Job drawing, mm, ordinate dimensions from the low corner. One solid piece. A direction names the side the tool comes from. Coordinates: 2 decimals unless noted, no trailing zeros. Write each loop counter-clockwise with the first axis right and the second up, starting at its lowest first coordinate (ties: lowest second). Pieces come first, ordered by that corner, then holes.
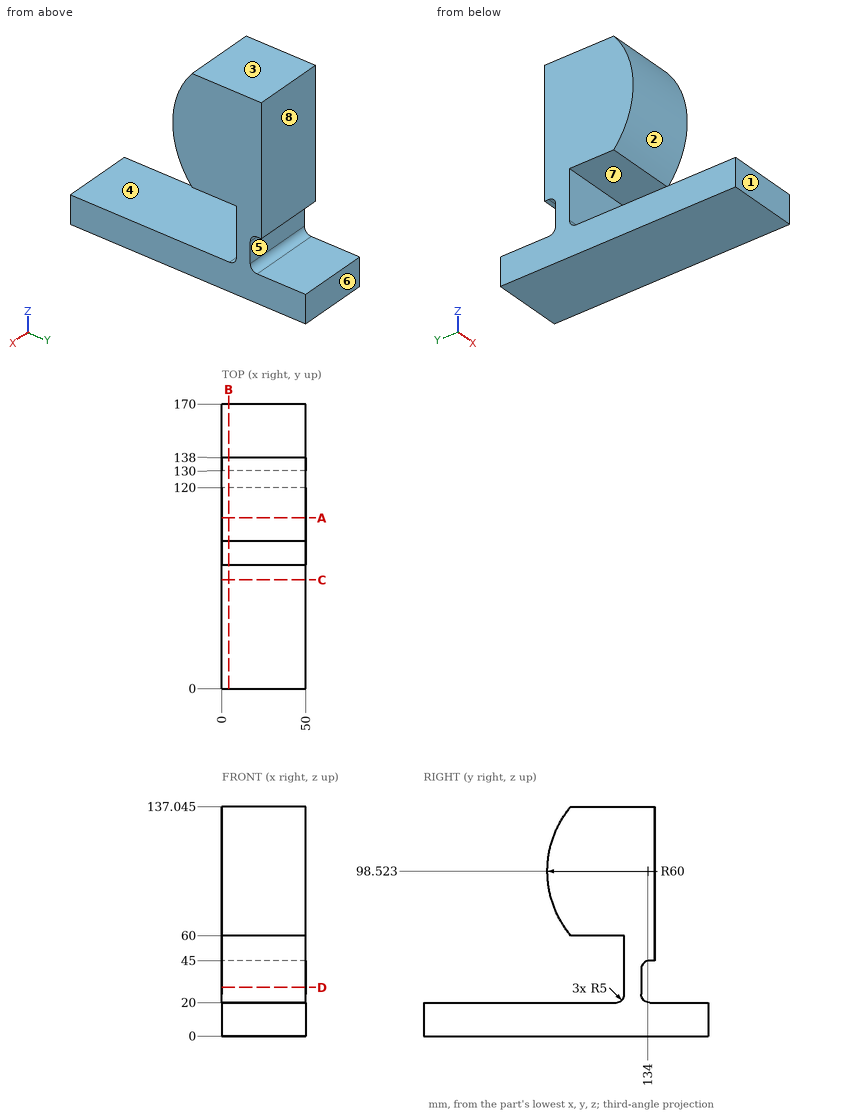
1. Saw through at D-D on z = 29. List the corners of the cut face in (x, y).
Computed values:
outline: (0, 120) - (50, 120) - (50, 130) - (0, 130) - close
2. Flat gauge pins, fed straight in: pin 1 (10.5 mm diameter, centred on x = 32.5, z = 38.5, fed in from -Y); pin 2 (16 mm diameter, centred on x = 35, y = 107.5, fed in from -Z); pin 3 (8 mm diameter, centred on x = 22, y = 36, fed in from +Z); pin 4 (25 mm diameter, centred on x = 14.5, y = 66.5, fed in from +Z) (1 decimal). Where does each tip first touch, or does it go through?
Computed values:
pin 1: stops at y = 120
pin 2: stops at z = 0
pin 3: stops at z = 20
pin 4: stops at z = 122.5
3. Mould opens along Z. For the marked faces 1, 2, 3 and 4 say: +Z half, -Z half, draft (parallel to the pull), parting line (faces both ways), or undercut.
Computed values:
face 1: draft
face 2: undercut
face 3: +Z half
face 4: undercut
4. 3-axis set-ups, long thin cutter, end or side, ignore diameter. For the marked faces 5, 6, 7 and 8: which of +Z, -Z, +X, -X, +Y, -Y reach the whole face in a straight line?
Computed values:
face 5: +X, -X, +Y
face 6: +Z, -Z, +X, -X, +Y
face 7: +X, -X, -Y
face 8: +Z, +X, -X, +Y
5. Probe line 1 along Z through (x, y) = (23.5, 101) (1 decimal); line 2 along Z through (x, y) = (18.5, 41); line 3 along Y through (x, z) = (3.5, 55). List the from-to ranges inside material, lowest first.
Computed values:
line 1: z = 0 to 20, 60 to 137
line 2: z = 0 to 20
line 3: y = 120 to 138
6. Saw through at C-C on y = 65. List the corners of the cut face in (x, z).
Computed values:
outline: (0, 0) - (50, 0) - (50, 20) - (0, 20) - close
7. Saw through at A-A on y = 102. List the corners of the cut face in (x, z) (1 decimal), plus the area to 3 significant figures.
Computed values:
outline: (0, 0) - (50, 0) - (50, 20) - (0, 20) - close; (0, 60) - (50, 60) - (50, 137) - (0, 137) - close
area: 4,850 mm2
8. Saw through at B-B on x = 4. List the corners of the cut face in (y, z) (1 decimal).
Computed values:
outline: (0, 0) - (170, 0) - (170, 20) - (135, 20) arc R5 cw to (130, 25) - (130, 40) arc R5 cw to (135, 45) - (138, 45) - (138, 137) - (88, 137) arc R60 ccw to (88, 60) - (120, 60) - (120, 25) arc R5 cw to (115, 20) - (0, 20) - close
